Model file for the job. Use its own axes, mm. Round coordinates to 2 decimals unless told otherwise and drop trailing zeros. Order: outer loops, then holes, each group sorted by start corner. A loop starts at its lowest first (then second) coordinate and runs counter-clockwise, first axis right, second up. Notation, with made-up numbers: (16, -4.75) - (58, -4.75) arc R13 ccw to (58, 1.25) - close; hole circle Ø10 at (24.25, 40.5). An arc over 180 degrees is marked (long way). Put each result on its own line as item: value. Start each with the question number.
Item 1: Pin check, flat tips, straight feed: pin 1 Ø1.5 at (y, z) = (4, 12) entering from -X; pin 2 Ø8 at (y, z) = (-11, 17) entering from +X. Stop position of each tip, or through.
Item 2: Probe probe 1 along Y at (x, z) = (0, 17.75); probe 2 along X at (y, z) = (1, 7.25); probe 3 along Y at (x, z) = (2, 8.5). List the from-to ranges inside material, lowest first.
Item 3: Mould opens along X. For faces 1 (the face through (-11.99, 0.53, 10.99)), 2 (the face through (-14.762, 8.683, 10.994)), 3 (the face through (-12, -4, 0)), 4 (the face through (8.92, 15.36, 22.13)) say: pulls with the +X half, pulls with the -X half, needs draft (parallel to the pull), parting line crosses it, or undercut.
Item 4: Saw through at A-A on z = 4.75. List the corners of the cut face in (x, y) (1 decimal).
```python
from build123d import *

# Parameters (mm, degrees)
SKETCH1_R          = 12
BASE_EXTRUDE_DEPTH = 22.3
SKETCH2_OUTSIDE_W  = 336.56
SKETCH2_OUTSIDE_H  = 331.262
SKETCH2_OUTSIDE_R  = 17.12565236
CUT_EXTRUDE1_DEPTH = 38
CUT_EXTRUDE1_DRAFT = -75
SKETCH3_OUTSIDE_W  = 336.56
SKETCH3_OUTSIDE_H  = 331.262
SKETCH3_OUTSIDE_R  = 17.12565236
CUT_EXTRUDE2_DEPTH = 38
CUT_EXTRUDE2_DRAFT = -75


with BuildPart() as part:
    # Sketch1 → Base-Extrude (new body)
    with BuildSketch(Plane.XY):
        Polygon((9.8875, 17.12565236), (-9.8875, 17.12565236), (-19.775, 0), (-9.8875, -17.12565236), (9.8875, -17.12565236), (19.775, 0), align=None)
        Circle(SKETCH1_R, mode=Mode.SUBTRACT)
    extrude(amount=BASE_EXTRUDE_DEPTH)


with BuildPart() as cut_extrude1_tool:
    # Sketch2 outside → Cut-Extrude1 (with draft: the straight prism first)
    with BuildSketch(Plane(origin=(0, 0, 0), x_dir=(-1, 0, 0), z_dir=(0, 0, -1))):
        Rectangle(SKETCH2_OUTSIDE_W, SKETCH2_OUTSIDE_H)
        Circle(SKETCH2_OUTSIDE_R, mode=Mode.SUBTRACT)
    extrude(amount=-CUT_EXTRUDE1_DEPTH)
    # Cut-Extrude1: the draft: its side faces are tilted about the plane it starts from
    cut_extrude1_sides = [cut_extrude1_tool.faces().sort_by_distance(p)[0] for p in [
        (0, -165.631, 19),
        (-168.28, 0, 19),
        (0, 165.631, 19),
        (168.28, 0, 19),
        (17.12565236, 0, 19),
    ]]
    draft(cut_extrude1_sides, Plane(origin=(0, 0, 0), x_dir=(-1, 0, 0), z_dir=(0, 0, -1)), CUT_EXTRUDE1_DRAFT)


with BuildPart() as part_1:
    add(part.part)

    # Cut-Extrude1: cut by cut_extrude1_tool
    add(cut_extrude1_tool.part, mode=Mode.SUBTRACT)


with BuildPart() as cut_extrude2_tool:
    # Sketch3 outside → Cut-Extrude2 (with draft: the straight prism first)
    with BuildSketch(Plane.XY.offset(22.3)):
        Rectangle(SKETCH3_OUTSIDE_W, SKETCH3_OUTSIDE_H)
        Circle(SKETCH3_OUTSIDE_R, mode=Mode.SUBTRACT)
    extrude(amount=-CUT_EXTRUDE2_DEPTH)
    # Cut-Extrude2: the draft: its side faces are tilted about the plane it starts from
    cut_extrude2_sides = [cut_extrude2_tool.faces().sort_by_distance(p)[0] for p in [
        (0, -165.631, 3.3),
        (168.28, 0, 3.3),
        (0, 165.631, 3.3),
        (-168.28, 0, 3.3),
        (-17.12565236, 0, 3.3),
    ]]
    draft(cut_extrude2_sides, Plane.XY.offset(22.3), CUT_EXTRUDE2_DRAFT)


with BuildPart() as part_2:
    add(part_1.part)

    # Cut-Extrude2: cut by cut_extrude2_tool
    add(cut_extrude2_tool.part, mode=Mode.SUBTRACT)


solid = part_2.part
```
Results found:
1. pin 1: stops at x = -17.9
1. pin 2: stops at x = 15.73
2. probe 1: y = -17.13 to -12, 12 to 17.13
2. probe 2: x = -19.2 to -11.96, 11.96 to 19.2
2. probe 3: y = -17.13 to -11.83, 11.83 to 17.13
3. face 1: undercut
3. face 2: pulls with the -X half
3. face 3: needs draft
3. face 4: pulls with the +X half
4. outline: (-19.8, 0) - (-9.9, -17.1) - (9.9, -17.1) - (19.8, 0) - (9.9, 17.1) - (-9.9, 17.1) - close; hole circle Ø24 at (0, 0)
